from build123d import *

# Parameters (mm, degrees)
SKETCH_1_W                  = 670
SKETCH_1_H                  = 280
SKETCH_1_W_2                = 590
SKETCH_1_H_2                = 200
EXTRUDE_1_DEPTH             = 4
HOLE_WIZARD_10_0_10_1_D     = 10
PATTERN_LINEAR_1_COUNT      = 5
PATTERN_LINEAR_1_PITCH      = 160
PATTERN_LINEAR_1_COUNT_DIR2 = 3
PATTERN_LINEAR_1_PITCH_DIR2 = 125


with BuildPart() as part:
    # 草图1 → 拉伸-薄壁1 (new body)
    with BuildSketch(Plane(origin=(0, 0, 0), x_dir=(0, 0, -1), z_dir=(1, 0, 0))):
        Rectangle(SKETCH_1_W, SKETCH_1_H)
        Rectangle(SKETCH_1_W_2, SKETCH_1_H_2, mode=Mode.SUBTRACT)
    extrude(amount=EXTRUDE_1_DEPTH)

    # Ø10.0 (10) 直径孔1 (through all)
    with Locations(Plane(origin=(4, 0, 0), x_dir=(0, 0, -1), z_dir=(1, 0, 0))):
        with Locations((-320, 125)):
            hole_wizard_10_0_10_1 = Hole(HOLE_WIZARD_10_0_10_1_D / 2)

    # 阵列(线性)1: Hole Wizard 10.0 _10_ _1 5 × 3, 3 skipped
    with Locations(*[(0, -j * PATTERN_LINEAR_1_PITCH_DIR2, -i * PATTERN_LINEAR_1_PITCH) for i in range(PATTERN_LINEAR_1_COUNT) for j in range(PATTERN_LINEAR_1_COUNT_DIR2) if (i, j) not in ((0, 0), (1, 1), (2, 1), (3, 1))]):
        add(hole_wizard_10_0_10_1, mode=Mode.SUBTRACT)


solid = part.part
The listing builds one solid part. Answer for the finished solid, in the listing's coordinates (mm). Give positions to 0.01 mm unless a question says otherwise; leave off trailing zeros. Write each loop counter-clockwise with the first axis right and the second up, starting at its lowest first coordinate (ties: lowest second). Pieces come first, ordered by that corner, then holes.
1) Section C-C (z = 82) is taken. Write down the section's boundary in (x, y).
2) Section B-B (x = 1.3) is taken. Count the separate pieces of the cut face and the enclosed holes in it, and give its area (3 significant figures).
3) Find the intervals of material crossed by L1, parallel to Y at x = 3.25, z = -160; L2, parallel to Z at x = 2.8, y = 48.5; L3, parallel to Y at x = 3.05, z = 285, in increasing order.
4) Section A-A (y = -74) is taken. Write down the section's boundary in (x, z), and give its area (3 significant figures).
5) Given P1, Ø13, axis at y = 0, z = -320, coming from the +X side; P2, Ø6, axis at y = 125, z = 320, coming from the +X side, each flat-ended and moving along its own axis, determine where each tip first touches the part or whether it passes through.
Response:
1. outline: (0, -140) - (4, -140) - (4, -100) - (0, -100) - close; (0, 100) - (4, 100) - (4, 140) - (0, 140) - close
2. separate pieces: 1
2. enclosed holes: 13
2. area: 68,700 mm2
3. L1: y = -140 to -130, -120 to -100, 100 to 120, 130 to 140
3. L2: z = -335 to -295, 295 to 335
3. L3: y = -140 to -100, 100 to 140
4. outline: (0, -335) - (4, -335) - (4, -295) - (0, -295) - close; (0, 295) - (4, 295) - (4, 335) - (0, 335) - close
4. area: 320 mm2
5. P1: stops at x = 4
5. P2: passes through
